from build123d import *

# Parameters (mm, degrees)
SKETCH1_R           = 2.5
BOSS_EXTRUDE1_DEPTH = 3


with BuildPart() as part:
    # Sketch1 → Boss-Extrude1 (new body)
    with BuildSketch(Plane.XY):
        with BuildLine():
            Line((4, 3), (61, 3))
            ThreePointArc((61, 3), (70, 0), (61, -3))
            Line((61, -3), (4, -3))
            ThreePointArc((4, -3), (-5, 0), (4, 3))
        make_face()
        Circle(SKETCH1_R, mode=Mode.SUBTRACT)
        with Locations((65, 0)):
            Circle(SKETCH1_R, mode=Mode.SUBTRACT)
    extrude(amount=BOSS_EXTRUDE1_DEPTH)


solid = part.part
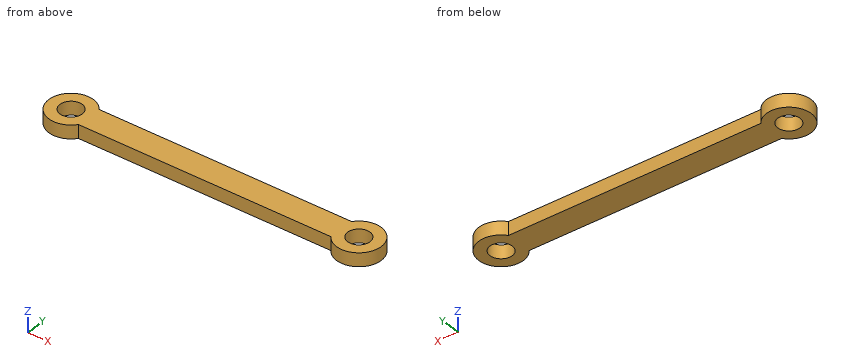
Can you work these out from the model? Positions are in its coordinate system, mm. Round coordinates to 2 decimals unless told otherwise and drop trailing zeros. Loops run counter-clockwise (first coordinate to the right, second up) from the corner with the lowest first, then second, coordinate; pieces in that order, holes last. Notation, with made-up numbers: (6.5, -8.5) - (50.5, -8.5) arc R29 ccw to (50.5, 18.5) - close; hole circle Ø2 at (-17, -4.75). An arc over 180 degrees is marked (long way). Write item = value, one per line. Start each with the question number.
(1) If we section it at C-C (y = 4): Please give me the cut outline in (x, z).
(2) If I drill on probe 1 along X at (y, z) = (-0.25, 2.4); probe 2 along Y at (x, z) = (0, 1.2); probe 3 along X at (y, z) = (-0.5, 1.7), over which ranges is the centre line in solid material (lowest first)? Write a range as [from, to].
(3) If we section it at A-A (y = 0): Please give me the cut outline in (x, z), and give its area (3 significant figures).
(4) For P1, Ø1, axis at y = -4, z = 2, coming from the -X side; P2, Ø4, axis at x = 65, y = 0, coming from the +Z side; P3, Ø0.9, axis at x = 33, z = 2, coming from the -Y side; P4, Ø0.9, axis at x = 19, z = 2, coming from the +Y side, each with a flat end and sliding along its axis, tell me the tip position at first contact or that it passes through.
(5) If we section it at D-D (z = 1.5): Please give me the cut outline in (x, y), and give its area (3 significant figures).
(6) If we section it at B-B (x = 65): Please give me the cut outline in (y, z), and give its area (3 significant figures).
Ans:
q1.outline = (-3, 0) - (3, 0) - (3, 3) - (-3, 3) - close; (62, 0) - (68, 0) - (68, 3) - (62, 3) - close
q2.probe_1 = [-4.99, -2.49], [2.49, 62.51], [67.49, 69.99]
q2.probe_2 = [-5, -2.5], [2.5, 5]
q2.probe_3 = [-4.97, -2.45], [2.45, 62.55], [67.45, 69.97]
q3.outline = (-5, 0) - (-2.5, 0) - (-2.5, 3) - (-5, 3) - close; (2.5, 0) - (62.5, 0) - (62.5, 3) - (2.5, 3) - close; (67.5, 0) - (70, 0) - (70, 3) - (67.5, 3) - close
q3.area = 195 mm²
q4.P1 = -3.57
q4.P2 = through
q4.P3 = -3
q4.P4 = 3
q5.outline = (4, -3) - (61, -3) arc R5 ccw (long way) to (61, 3) - (4, 3) arc R5 ccw (long way) to start; hole circle Ø5 at (0, 0); hole circle Ø5 at (65, 0)
q5.area = 452 mm²
q6.outline = (-5, 0) - (-2.5, 0) - (-2.5, 3) - (-5, 3) - close; (2.5, 0) - (5, 0) - (5, 3) - (2.5, 3) - close
q6.area = 15.0 mm²
